```python
from build123d import *

# Parameters (mm, degrees)
BASE_PLATE_DEPTH            = 30
SIDE_LUG_DEPTH              = 26
GUIDE_RAIL_PROFILE_DEPTH    = 165
END_BLOCK_SKETCH_W          = 26
END_BLOCK_SKETCH_H          = 67
END_BLOCK_DEPTH             = 30
END_NOTCH_SKETCH_W          = 19
END_NOTCH_SKETCH_H          = 14
END_NOTCH_SKETCH_W_2        = 32
END_NOTCH_CUT_DEPTH         = 26
NOTCH_FILLET_R1_5_A_R       = 1.5
NOTCH_FILLET_R1_5_B_R       = 1.5
MOUNTING_HOLE_SKETCH_R      = 6
MOUNTING_HOLE_DEPTH_8_DEPTH = 8
THROUGH_HOLE_SKETCH_R       = 3.5
THROUGH_HOLE_DEPTH_32_DEPTH = 32
END_BLOCK_FILLET_R8_R       = 8
SIDE_LUG_FILLET_R8_R        = 8
LONG_BORE_A_SKETCH_R        = 3.5
LONG_BORE_A_DEPTH_96_DEPTH  = 96
LONG_BORE_B_SKETCH_R        = 3.53
LONG_BORE_B_DEPTH_96_DEPTH  = 96
CENTRE_BOSS_SKETCH_W        = 22
CENTRE_BOSS_SKETCH_H        = 38
CENTRE_BOSS_DEPTH           = 14
CENTRE_SLOT_CUT_DEPTH       = 14
COUNTERBORE_10_SKETCH_R     = 5
COUNTERBORE_10_DEPTH        = 8
DEEP_BORE_SKETCH_R          = 4
DEEP_BORE_DEPTH_65_DEPTH    = 65
SECOND_END_NOTCH_SKETCH_W   = 32
SECOND_END_NOTCH_SKETCH_H   = 14
SECOND_END_NOTCH_SKETCH_W_2 = 19
SECOND_END_NOTCH_CUT_DEPTH  = 26


with BuildPart() as part:
    # Base Plate Sketch → Base Plate (new body)
    with BuildSketch(Plane(origin=(0, 0, 0), x_dir=(1, 0, 0), z_dir=(0, 1, 0))):
        Polygon((44, 0), (44, -82.5), (-44, -82.5), (-44, 82.5), (44, 82.5), align=None)
    extrude(amount=-BASE_PLATE_DEPTH)

    # Side Lug Sketch → Side Lug (add)
    with BuildSketch(Plane(origin=(44, 0, 0), x_dir=(0, 0, -1), z_dir=(1, 0, 0))):
        Polygon((-82.5, -30), (-82.5, 0), (-44.5, 0), (-44.5, -16), (-66.5, -16), (-66.5, -30), align=None)
    side_lug = extrude(amount=SIDE_LUG_DEPTH)

    # Side Lug Mirror: Side Lug across plane
    add(side_lug.mirror(Plane(origin=(0, 0, 0), x_dir=(0, 0, 1), z_dir=(1, 0, 0))))


with BuildPart() as guide_rail_profile_tool:
    # Guide Rail Profile Sketch → Guide Rail Profile (new body)
    with BuildSketch(Plane.XY.offset(82.5)):
        with BuildLine():
            Line((11, 14), (11, 0))
            Line((11, 0), (44, 0))
            Line((44, 0), (44, 2.5))
            ThreePointArc((44, 2.5), (43.560660172, 3.560660172), (42.5, 4))
            Line((42.5, 4), (22.92116461, 4))
            ThreePointArc((22.92116461, 4), (21.738856453, 4.576881686), (21.465950859, 5.863803438))
            Line((21.465950859, 5.863803438), (23.034049141, 12.136196562))
            ThreePointArc((23.034049141, 12.136196562), (22.761143547, 13.423118314), (21.57883539, 14))
            Line((21.57883539, 14), (11, 14))
        make_face()
        with BuildLine():
            Line((-44, 7.32e-07), (-11, 0))
            Line((-11, 0), (-11, 14))
            Line((-11, 14), (-21.57883539, 14))
            ThreePointArc((-21.57883539, 14), (-22.761143547, 13.423118314), (-23.034049141, 12.136196562))
            Line((-23.034049141, 12.136196562), (-21.465950859, 5.863803438))
            ThreePointArc((-21.465950859, 5.863803438), (-21.738856678, 4.576881398), (-22.921165341, 4))
            Line((-22.921165341, 4), (-42.500000732, 4))
            ThreePointArc((-42.500000732, 4), (-43.560660172, 3.560660172), (-44, 2.500000732))
            Line((-44, 2.500000732), (-44, 7.32e-07))
        make_face()
    extrude(amount=-GUIDE_RAIL_PROFILE_DEPTH)


with BuildPart() as part_1:
    add(part.part)


with BuildPart() as part_2:
    # Guide Rail Profile: joined with guide_rail_profile_tool
    add(part_1.part.fuse(guide_rail_profile_tool.part, tol=0.00001))

    # End Block Sketch → End Block (add)
    with BuildSketch(Plane(origin=(0, 0, 0), x_dir=(1, 0, 0), z_dir=(0, 1, 0))):
        with Locations((-57, 49)):
            Rectangle(END_BLOCK_SKETCH_W, END_BLOCK_SKETCH_H)
    end_block = extrude(amount=-END_BLOCK_DEPTH)

    # End Notch Sketch → End Notch Cut (cut)
    with BuildSketch(Plane.ZY.offset(70)):
        with Locations((-25, -23)):
            Rectangle(END_NOTCH_SKETCH_W, END_NOTCH_SKETCH_H)
        with Locations((-66.5, -23)):
            Rectangle(END_NOTCH_SKETCH_W_2, END_NOTCH_SKETCH_H)
    end_notch_cut = extrude(amount=-END_NOTCH_CUT_DEPTH, mode=Mode.SUBTRACT)

    # Notch Fillet R1.5 A
    notch_fillet_r1_5_a_edges = [part_2.edges().sort_by_distance(p)[0] for p in [
        (-57, -16, -50.5),
    ]]
    fillet(notch_fillet_r1_5_a_edges, radius=NOTCH_FILLET_R1_5_A_R)

    # Notch Fillet R1.5 B
    notch_fillet_r1_5_b_edges = [part_2.edges().sort_by_distance(p)[0] for p in [
        (-57, -16, -34.5),
    ]]
    fillet(notch_fillet_r1_5_b_edges, radius=NOTCH_FILLET_R1_5_B_R)

    # Mounting Hole Sketch → Mounting Hole Depth 8 (cut)
    with BuildSketch(Plane(origin=(0, 0, 0), x_dir=(1, 0, 0), z_dir=(0, 1, 0))):
        with Locations(Location((-59.808082778, 72.5, 0), (0, 0, 270))):
            Circle(MOUNTING_HOLE_SKETCH_R)
    mounting_hole_depth_8 = extrude(amount=-MOUNTING_HOLE_DEPTH_8_DEPTH, mode=Mode.SUBTRACT)

    # Through Hole Sketch → Through Hole Depth 32 (cut)
    with BuildSketch(Plane(origin=(0, 0, 0), x_dir=(1, 0, 0), z_dir=(0, 1, 0))):
        with Locations(Location((-59.808082778, 72.5, 0), (0, 0, 270))):
            Circle(THROUGH_HOLE_SKETCH_R)
    extrude(amount=-THROUGH_HOLE_DEPTH_32_DEPTH, mode=Mode.SUBTRACT)

    # Mounting Hole Mirror: End Block, Mounting Hole Depth 8 across plane
    add(end_block.mirror(Plane(origin=(0, 0, 0), x_dir=(0, 0, 1), z_dir=(1, 0, 0))))
    add(mounting_hole_depth_8.mirror(Plane(origin=(0, 0, 0), x_dir=(0, 0, 1), z_dir=(1, 0, 0))), mode=Mode.SUBTRACT)

    # End Block Fillet R8
    end_block_fillet_r8_edges = [part_2.edges().sort_by_distance(p)[0] for p in [
        (-44, -8, -15.5),
    ]]
    fillet(end_block_fillet_r8_edges, radius=END_BLOCK_FILLET_R8_R)

    # Side Lug Fillet R8
    side_lug_fillet_r8_edges = [part_2.edges().sort_by_distance(p)[0] for p in [
        (-44, -8, 44.5),
    ]]
    fillet(side_lug_fillet_r8_edges, radius=SIDE_LUG_FILLET_R8_R)

    # Body Mirror: part across plane


with BuildPart() as part_3:
    add(part_2.part)
    add(part_2.part.mirror(Plane(origin=(0, 0, 0), x_dir=(0, 0, 1), z_dir=(1, 0, 0))))

    # Long Bore A Sketch → Long Bore A Depth 96 (cut)
    with BuildSketch(Plane(origin=(0, -8, 0), x_dir=(1, 0, 0), z_dir=(0, 1, 0))):
        with Locations(Location((-59.808082778, 72.5, 0), (0, 0, 270))):
            Circle(LONG_BORE_A_SKETCH_R)
    long_bore_a_depth_96 = extrude(amount=-LONG_BORE_A_DEPTH_96_DEPTH, mode=Mode.SUBTRACT)

    # Long Bore B Sketch → Long Bore B Depth 96 (cut)
    with BuildSketch(Plane.XZ.offset(30)):
        with Locations(Location((59.808082778, -72.5, 0), (0, 0, 270))):
            Circle(LONG_BORE_B_SKETCH_R)
    extrude(amount=-LONG_BORE_B_DEPTH_96_DEPTH, mode=Mode.SUBTRACT)

    # Centre Boss Sketch → Centre Boss (add)
    with BuildSketch(Plane(origin=(0, 14, 0), x_dir=(1, 0, 0), z_dir=(0, 1, 0))):
        with Locations((0, 63.5)):
            Rectangle(CENTRE_BOSS_SKETCH_W, CENTRE_BOSS_SKETCH_H)
    extrude(amount=-CENTRE_BOSS_DEPTH)

    # Centre Slot Sketch → Centre Slot Cut (cut)
    with BuildSketch(Plane(origin=(0, 14, 0), x_dir=(1, 0, 0), z_dir=(0, 1, 0))):
        with BuildLine():
            Line((-11, 44.5), (11, 44.5))
            ThreePointArc((11, 44.5), (0, 55.5), (-11, 44.5))
        make_face()
    extrude(amount=-CENTRE_SLOT_CUT_DEPTH, mode=Mode.SUBTRACT)

    # Counterbore Ø10 Sketch → Counterbore Ø10 (cut)
    with BuildSketch(Plane(origin=(0, 0, 0), x_dir=(1, 0, 0), z_dir=(0, 1, 0))):
        with Locations(Location((0, -58.5, 0), (0, 0, 270))):
            Circle(COUNTERBORE_10_SKETCH_R)
    extrude(amount=-COUNTERBORE_10_DEPTH, mode=Mode.SUBTRACT)

    # Deep Bore Sketch → Deep Bore Depth 65 (cut)
    with BuildSketch(Plane(origin=(0, -8, 0), x_dir=(1, 0, 0), z_dir=(0, 1, 0))):
        with Locations(Location((0, -58.5, 0), (0, 0, 270))):
            Circle(DEEP_BORE_SKETCH_R)
    extrude(amount=-DEEP_BORE_DEPTH_65_DEPTH, mode=Mode.SUBTRACT)

    # Second End Notch Sketch → Second End Notch Cut (cut)
    with BuildSketch(Plane.ZY.offset(70)):
        with Locations((-31.5, -23)):
            Rectangle(SECOND_END_NOTCH_SKETCH_W, SECOND_END_NOTCH_SKETCH_H)
        with Locations((-73, -23)):
            Rectangle(SECOND_END_NOTCH_SKETCH_W_2, SECOND_END_NOTCH_SKETCH_H)
    extrude(amount=-SECOND_END_NOTCH_CUT_DEPTH, mode=Mode.SUBTRACT)

    # End Notch Mirror: End Block, End Notch Cut across plane
    add(end_block.mirror(Plane(origin=(0, 0, 0), x_dir=(0, 0, 1), z_dir=(1, 0, 0))))
    add(end_notch_cut.mirror(Plane(origin=(0, 0, 0), x_dir=(0, 0, 1), z_dir=(1, 0, 0))), mode=Mode.SUBTRACT)

    # Mounting Hole Mirror 2: Mounting Hole Depth 8 across plane
    add(mounting_hole_depth_8.mirror(Plane(origin=(0, 0, 0), x_dir=(0, 0, 1), z_dir=(1, 0, 0))), mode=Mode.SUBTRACT)

    # Long Bore Mirror: Long Bore A Depth 96 across plane
    add(long_bore_a_depth_96.mirror(Plane(origin=(0, 0, 0), x_dir=(0, 0, 1), z_dir=(1, 0, 0))), mode=Mode.SUBTRACT)


solid = part_3.part
```
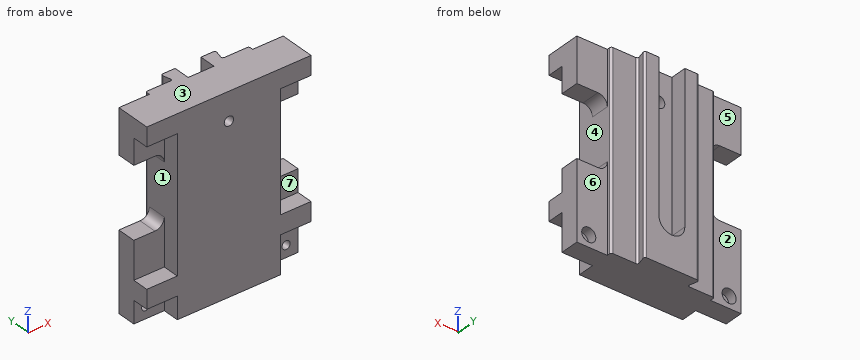
Work out the finished part from the listing and answer in its coordinate system (mm). Face numbers are marked on the shaded views. A direction names the side the tool comes from. Give positions to 0.01 mm unless a question says otherwise; leave off trailing zeros. Order: outer loops, then holes, each group sorted by start corner. A loop starts at its lowest first (then second) coordinate and runs counter-clockwise, first axis right, second up. Notation, with made-up numbers: (87.5, 74.5) - (101.5, 74.5) arc R19 ccw to (101.5, 81.5) - close; hole circle Ø1 at (-4, 56.25). An arc over 180 degrees is marked (long way). One line per item, written item: value. Start each with the question number.
1. Which of the six approach directions +Z, -Z, +X, -X, +Y, -Y give full straight-line access (tool end or side, diameter ignored) to the marked faces 4, 5, 6 and 7?
2. Section B-B, the plane y = -27 is taken. Write down the section's boundary in (x, z).
3. Each of these flat-tipped pins is pushed along its axis until it touches: pin 1 Ø24 at (x, z) = (-3.5, 25) entering from +Y; pin 2 Ø11 at (x, y) = (52, -22.5) entering from -Z; pin 3 Ø6 at (y, z) = (-23.5, -18.5) entering from +X; pin 4 Ø10 at (x, z) = (-37, 32.5) entering from +Y. Where does it stop, or does it pass through?
4. Consider line 1 (X direction, y = -5, z = -72); line 2 (X direction, y = -10.5, z = -72.5); line 3 (X direction, y = -4, z = 58). Determine where each line is inside the solid, lowest interval first.
5. Section C-C, the plane x = 0 is taken. Write down the section's boundary in (y, z), then the cut area to 3 significant figures.
6. For a pull along Z with two mould halves and no side action, classify the marked faces 1, 2 and 3 as released by +Z, released by -Z, zero draft, split by the parting line, or undercut.
Filled sheet:
1. face 4: +X
1. face 5: +Z, -Z, -X, +Y
1. face 6: +Z, -Z, +X, +Y
1. face 7: +X, -Y
2. outline: (-70, -63.5) - (-44, -63.5) - (-44, -82.5) - (44, -82.5) - (44, -50.5) - (70, -50.5) - (70, -34.5) - (44, -34.5) - (44, 66.5) - (70, 66.5) - (70, 82.5) - (-70, 82.5) - (-70, 66.5) - (-44, 66.5) - (-44, -47.5) - (-70, -47.5) - close; hole circle Ø8 at (0, 58.5)
3. pin 1: y = 14
3. pin 2: z = -50.5
3. pin 3: x = 44
3. pin 4: y = 4
4. line 1: -70 to -65.79, -53.83 to 53.83, 65.79 to 70
4. line 2: -70 to -63.31, -56.31 to 56.31, 63.31 to 70
4. line 3: -70 to -4.97, 4.97 to 70
5. outline: (-30, -82.5) - (14, -82.5) - (14, -55.5) - (0, -55.5) - (0, 53.5) - (-8, 53.5) - (-8, 54.5) - (-30, 54.5) - close; (-30, 62.5) - (-8, 62.5) - (-8, 63.5) - (0, 63.5) - (0, 82.5) - (-30, 82.5) - close
5. area: 5,070 mm²
6. face 1: undercut
6. face 2: zero draft
6. face 3: released by +Z
